Here's the drawing with two shaded views (mm, measured from the low corner). I have some questions. A direction names the side the tool comes from. Round coordinates to 2 decimals unless told otherwise and drop trailing zeros. Write each loop counter-clockwise with the first axis right and the second up, starting at its lowest first coordinate (ties: lowest second). Pieces come first, ordered by that corner, then holes. Notation, with made-up numbers: M -29,-4.5 L 27,-4.5 A36 ccw 27,31.5 Z; hole C 34,29.25 d9. An arc over 180 degrees is marked long. Use one line per item in the form item = value. Start each with the question number.
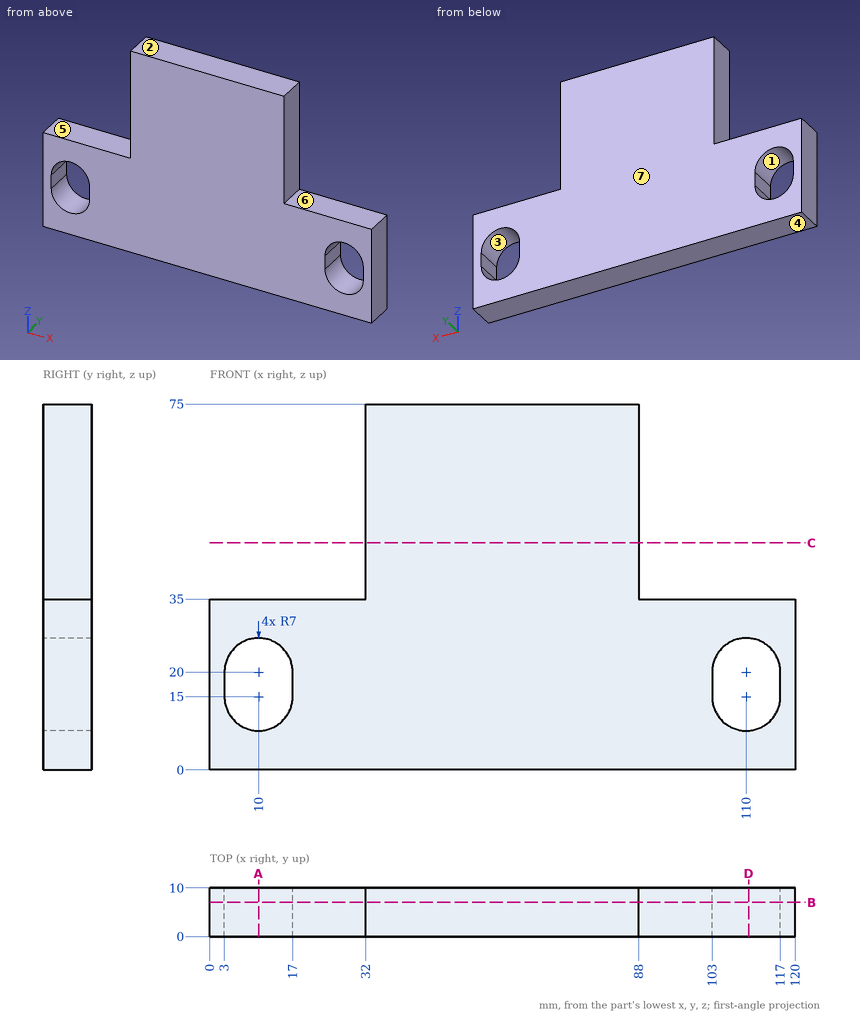
1. If we section it at B-B (y = 7): List the corners of the cut face in (x, z) for me, and give its area (3 significant figures).
2. Please list where these lines run through material, in increasing order: line 1 along Z through (x, y) = (110, 6); line 2 along X through (y, z) = (2.25, 25); line 3 along Z through (x, y) = (23.5, 9.75).
3. If we section it at A-A (x = 10): List the corners of the cut face in (y, z) for me.
4. Which directions (+Z, -Z, +X, -X, +Y, -Y) give clear straight access to the entire face, cutting with the end or side of a thin tool? Please do the marked faces 3, 4, 5, 6 and 7.
5. If we mould it in two halves opening along X, with no side actions, what happens to the marked faces 1 and 2? For each: pulls with the +X half, pulls with the -X half, needs draft (parallel to the pull), parting line crosses it, or undercut.
6. If we section it at D-D (x = 110.5): List the corners of the cut face in (y, z) for me, and give its area (3 significant figures).
7. If we section it at C-C (z = 46.5): List the corners of the cut face in (x, y) for me.
8. Will these pins go through, and if not, where does the flat tip stop? pin 1 (3 mm diameter, centred on x = 104.5, y = 3, fed in from +Z); pin 2 (6 mm diameter, centred on y = 8, z = 65.5, fed in from +X).
Model answer:
q1.outline = M 0,0 L 120,0 L 120,35 L 88,35 L 88,75 L 32,75 L 32,35 L 0,35 Z; hole M 3,15 A7 ccw 17,15 L 17,20 A7 ccw 3,20 Z; hole M 103,15 A7 ccw 117,15 L 117,20 A7 ccw 103,20 Z
q1.area = 5,990 mm2
q2.line_1 = 0 to 8, 27 to 35
q2.line_2 = 0 to 5.1, 14.9 to 105.1, 114.9 to 120
q2.line_3 = 0 to 35
q3.outline = M 0,0 L 10,0 L 10,8 L 0,8 Z; M 0,27 L 10,27 L 10,35 L 0,35 Z
q4.face_3 = +Y, -Y
q4.face_4 = -Z, +X, -X, +Y, -Y
q4.face_5 = +Z, -X, +Y, -Y
q4.face_6 = +Z, +X, +Y, -Y
q4.face_7 = +Z, -Z, +X, -X, +Y
q5.face_1 = undercut
q5.face_2 = needs draft
q6.outline = M 0,0 L 10,0 L 10,8.02 L 0,8.02 Z; M 0,26.98 L 10,26.98 L 10,35 L 0,35 Z
q6.area = 160 mm2
q7.outline = M 32,0 L 88,0 L 88,10 L 32,10 Z
q8.pin_1 = 35
q8.pin_2 = 88
